from build123d import *

# Parameters (mm, degrees)
BASEHEAD_DEPTH = 7.68
SKETCH5_R      = 6
BASEBODY_DEPTH = 30
CHAMFER1_SIZE  = 0.6


with BuildPart() as part:
    # Sketch2 → BaseHead (new body)
    with BuildSketch(Plane(origin=(0, 0, 0), x_dir=(0, 0, -1), z_dir=(1, 0, 0))):
        Polygon((8.865, -5.118210136), (8.865, 5.118210136), (0, 10.236420273), (-8.865, 5.118210136), (-8.865, -5.118210136), (0, -10.236420273), align=None)
    extrude(amount=BASEHEAD_DEPTH)

    # Sketch3 → BearingFace (revolve, cut)
    with BuildSketch(Plane.XY, mode=Mode.PRIVATE) as bearingface_sk:
        Polygon((7.68, 10.236420273), (7.68, 8.315), (7.08, 8.915), (7.08, 10.236420273), align=None)
    revolve(bearingface_sk.sketch.rotate(Axis((-0.957090588, 0, 0), (1, 0, 0)), 90), axis=Axis((-0.957090588, 0, 0), (1, 0, 0)), mode=Mode.SUBTRACT)

    # Sketch4 → HeadChamfer (revolve, cut)
    with BuildSketch(Plane.XY):
        Polygon((0, 10.236420273), (0.499156158, 10.236420273), (0, 8.865), align=None)
    revolve(axis=Axis((-0.493528746, 0, 0), (1, 0, 0)), mode=Mode.SUBTRACT)

    # Sketch5 → BaseBody (add)
    with BuildSketch(Plane(origin=(7.68, 0, 0), x_dir=(0, 0, -1), z_dir=(1, 0, 0))):
        Circle(SKETCH5_R)
    extrude(amount=BASEBODY_DEPTH)

    # Chamfer1
    chamfer1_edges = [part.edges().sort_by_distance(p)[0] for p in [
        (37.68, 0, 6),
    ]]
    chamfer(chamfer1_edges, length=CHAMFER1_SIZE)


solid = part.part
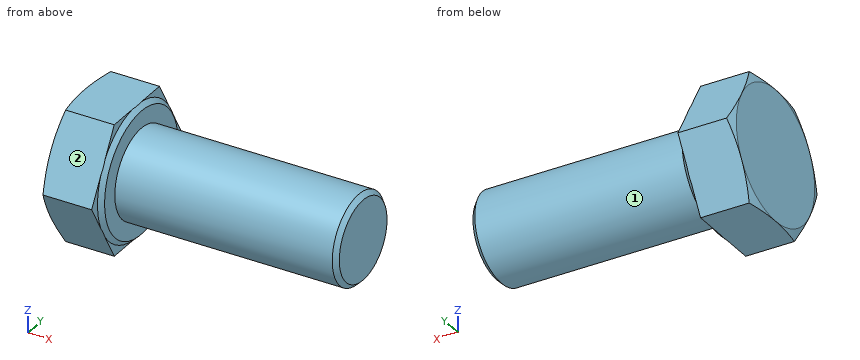
Could you check a few things on this model? Use its own coordinates, in mm. Face numbers are marked on the shaded views. A direction names the side the tool comes from. Give positions to 0.01 mm unless a question says otherwise; leave off trailing zeros. Loops run counter-clockwise (first coordinate to the right, second up) from the corner with the lowest first, then second, coordinate; pieces in that order, holes last. Notation, with made-up numbers: (13, -34.75) -> (65, -34.75) arc R27 cw to (65, -0.75) -> close; hole circle Ø2 at (18.25, 13.25). An arc over 180 degrees is marked (long way). Answer as CSV lines item,"result". Start each with the question number.
(1) If we section it at A-A on x = 16.5: Write out the boundary of the cut face in (y, z).
(2) I'm going to push flat-ended pins straight in: pin 1 Ø4 at (y, z) = (5.5, 6) entering from +X; pin 2 Ø1 at (y, z) = (9, -1) entering from +X; pin 3 Ø2 at (x, z) = (28, -4.5) entering from +Y. Where does each tip first touch, or does it pass through?
(3) I need wall thicknesses on probe 1 along X at (y, z) = (-2.5, 6); probe 2 along Z at (x, y) = (31, -0.25); probe 3 along X at (y, z) = (5, 7.25). Which ranges of each line are inside material? Lowest first, please.
(4) Which directions (+Z, -Z, +X, -X, +Y, -Y) give clear straight access to the entire face, cutting with the end or side of a thin tool? Please do the marked faces 1 and 2.
Computed:
1,outline,"circle Ø12 at (0, 0)"
2,pin 1,"stops at x = 7.68"
2,pin 2,"stops at x = 7.44"
2,pin 3,"stops at y = 4.87"
3,probe 1,"x = 0 to 7.68"
3,probe 2,"z = -5.99 to 5.99"
3,probe 3,"x = 0 to 7.19"
4,face 1,"+X"
4,face 2,"+Z, +X, -X, -Y"
